Part model, mm, in its own coordinate system. Face numbers are marked on the shaded views. Round coordinates to 2 decimals unless told otherwise and drop trailing zeros. Order: outer loops, then holes, each group sorted by start corner. A loop starts at its lowest first (then second) coordinate and runs counter-clockwise, first axis right, second up. Notation, with made-up numbers: (45.5, 24.25) - (81.5, 24.25) arc R22 ccw to (81.5, 63.25) - close; hole circle Ø6 at (34.5, -34). An arc over 180 degrees is marked (long way). Answer as a JSON object with one key per item and string values.
```python
from build123d import *

# Parameters (mm, degrees)
SKETCH1_W                                         = 600
SKETCH1_H                                         = 195
EXTRUDE1_DEPTH                                    = 6
CHAMFER1_SIZE                                     = 5
M6_SOCKET_HEAD_CAP_SCREW_COUNTERBORE1_D           = 6.6
M6_SOCKET_HEAD_CAP_SCREW_COUNTERBORE1_CBORE_D     = 11
M6_SOCKET_HEAD_CAP_SCREW_COUNTERBORE1_CBORE_DEPTH = 7
M4_TAPPED_HOLE1_D                                 = 3.3
M4_TAPPED_HOLE1_DEPTH                             = 10.1
M4_TAPPED_HOLE1_TIP                               = 0.991420021
M8_TAPPED_HOLE1_D                                 = 6.8
M6_TAPPED_HOLE2_D                                 = 5
SKETCH10_R                                        = 20
CUT_EXTRUDE1_DEPTH                                = 316.674278331
SKETCH11_R                                        = 10
CUT_EXTRUDE2_DEPTH                                = 316.674278331
M4_TAPPED_HOLE2_D                                 = 3.3
M4_TAPPED_HOLE2_DEPTH                             = 12
M4_TAPPED_HOLE2_TIP                               = 0.991420021
SKETCH13_R                                        = 5
CUT_EXTRUDE3_DEPTH                                = 316.674278331


with BuildPart() as part:
    # Sketch1 → Extrude1 (new, symmetric)
    with BuildSketch(Plane(origin=(0, 0, 0), x_dir=(1, 0, 0), z_dir=(0, 1, 0))):
        Rectangle(SKETCH1_W, SKETCH1_H)
    extrude(amount=EXTRUDE1_DEPTH, both=True)

    # Chamfer1
    chamfer1_edges = [part.edges().sort_by_distance(p)[0] for p in [
        (-300, 0, -97.5),
        (300, 0, -97.5),
    ]]
    chamfer(chamfer1_edges, length=CHAMFER1_SIZE)

    # M6 Socket Head Cap Screw Counterbore1 (through all)
    with Locations(Plane(origin=(-280, 6, -77.5), x_dir=(0, 0, 1), z_dir=(0, 1, 0))):
        with Locations((0, 0), (100, 0), (0, 480), (0, 560), (150, 560), (150, 480)):
            CounterBoreHole(M6_SOCKET_HEAD_CAP_SCREW_COUNTERBORE1_D / 2, M6_SOCKET_HEAD_CAP_SCREW_COUNTERBORE1_CBORE_D / 2, M6_SOCKET_HEAD_CAP_SCREW_COUNTERBORE1_CBORE_DEPTH)

    # M4 Tapped Hole1
    with Locations(Plane(origin=(-230, 0, 97.5), x_dir=(1, 0, 0), z_dir=(0, 0, 1))):
        with Locations((0, 0), (250, 0), (500, 0)):
            Hole(M4_TAPPED_HOLE1_D / 2, depth=M4_TAPPED_HOLE1_DEPTH)
            with Locations((0, 0, -(M4_TAPPED_HOLE1_DEPTH + M4_TAPPED_HOLE1_TIP / 2))):  # 118° drill point
                Cone(0, M4_TAPPED_HOLE1_D / 2, M4_TAPPED_HOLE1_TIP, mode=Mode.SUBTRACT)

    # M8 Tapped Hole1 (through all)
    with Locations(Plane(origin=(-174, 6, 81.5), x_dir=(0, 0, 1), z_dir=(0, 1, 0))):
        with Locations((0, 0), (0, 50), (-55, 50), (-55, 0)):
            Hole(M8_TAPPED_HOLE1_D / 2)

    # M6 Tapped Hole2 (through all)
    with Locations(Plane(origin=(55, 6, -77.5), x_dir=(0, 0, 1), z_dir=(0, 1, 0))):
        with Locations((0, 0), (0, -250)):
            Hole(M6_TAPPED_HOLE2_D / 2)

    # Sketch10 → Cut-Extrude1 (cut, through all)
    with BuildSketch(Plane(origin=(0, 6, 0), x_dir=(1, 0, 0), z_dir=(0, 1, 0))):
        with Locations(Location((-230, -27.5, 0), (0, 0, 270))):
            Circle(SKETCH10_R)
    extrude(amount=-CUT_EXTRUDE1_DEPTH, mode=Mode.SUBTRACT)

    # Sketch11 → Cut-Extrude2 (cut, through all)
    with BuildSketch(Plane(origin=(0, 6, 0), x_dir=(1, 0, 0), z_dir=(0, 1, 0))):
        with Locations(Location((100, 47.5, 0), (0, 0, 270))):
            Circle(SKETCH11_R)
    extrude(amount=-CUT_EXTRUDE2_DEPTH, mode=Mode.SUBTRACT)

    # M4 Tapped Hole2
    with Locations(Plane(origin=(-25, 6, 47.5), x_dir=(0, 0, 1), z_dir=(0, 1, 0))):
        with Locations((0, 0), (-25, 0)):
            Hole(M4_TAPPED_HOLE2_D / 2, depth=M4_TAPPED_HOLE2_DEPTH)
            with Locations((0, 0, -(M4_TAPPED_HOLE2_DEPTH + M4_TAPPED_HOLE2_TIP / 2))):  # 118° drill point
                Cone(0, M4_TAPPED_HOLE2_D / 2, M4_TAPPED_HOLE2_TIP, mode=Mode.SUBTRACT)

    # Sketch13 → Cut-Extrude3 (cut, through all)
    with BuildSketch(Plane(origin=(0, 6, 0), x_dir=(1, 0, 0), z_dir=(0, 1, 0))):
        with Locations(Location((-45, -35.825, 0), (0, 0, 270))):
            Circle(SKETCH13_R)
    extrude(amount=-CUT_EXTRUDE3_DEPTH, mode=Mode.SUBTRACT)


solid = part.part
```
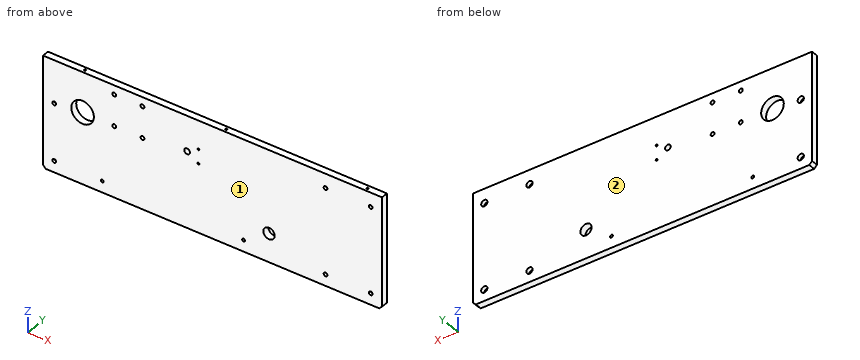
Item 1: Drop a flat-ended pin along its axis: P1, Ø8.5, axis at x = 280, z = 72.5, coming from the +Y side. Give the stop position or say it passes through.
Taken from the geometry:
{"P1": "y = -1"}
Item 2: Two-plate mould, pull along Y, no slides. Class the marked faces 1 and 2: pulls with the +Y half, pulls with the -Y half, needs draft (parallel to the pull), parting line crosses it, or undercut.
Taken from the geometry:
{"face 1": "pulls with the -Y half", "face 2": "pulls with the +Y half"}
Item 3: Cut at B-B (x = 100). Write the cut outline in (y, z), plus the area to 3 significant figures.
Taken from the geometry:
{"outline": "(-6, -97.5) - (6, -97.5) - (6, -57.5) - (-6, -57.5) - close; (-6, -37.5) - (6, -37.5) - (6, 97.5) - (-6, 97.5) - close", "area": "2,100 mm2"}
Item 4: Probe L1, parallel to X at y = -1.75, z = 73; L2, parallel to X at y = 3.25, z = -77.5; L3, parallel to Z at x = -124.5, y = -0.5. List the from-to ranges inside material, lowest first. Write a range as from..to.
Taken from the geometry:
{"L1": "-300..196.74, 203.26..276.74, 283.26..300", "L2": "-300..-285.5, -274.5..-197.5, -192.5..52.5, 57.5..194.5, 205.5..274.5, 285.5..300", "L3": "-97.5..23.14, 29.86..78.14, 84.86..97.5"}
Item 5: Cut at A-A (z = -47.5). Write the cut outline in (x, y), plus the area to 3 significant figures.
Taken from the geometry:
{"outline": "(-300, -6) - (90, -6) - (90, 6) - (-300, 6) - close; (110, -6) - (300, -6) - (300, 6) - (110, 6) - close", "area": "6,960 mm2"}
